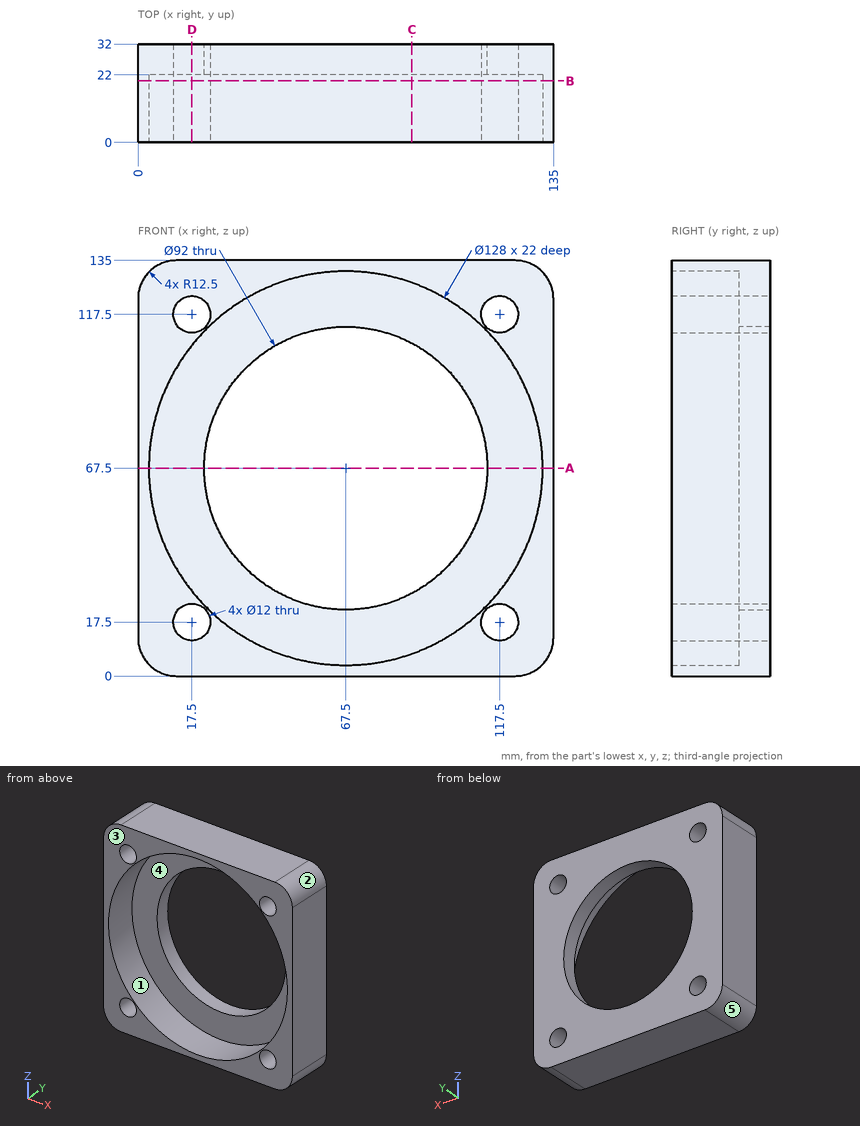
Check sheet for the drawn part. Datum: minimum x, y, z corner. Units: mm. A direction names the side the tool comes from. Give positions to 0.01 mm unless a question says otherwise; leave off trailing zeros. Order: outer loops, then holes, each group sorted by start corner. A loop starts at its lowest first (then second) coordinate and runs counter-clockwise, first axis right, second up. Notation, with made-up numbers: (32, -35.75) -> (85, -35.75) arc R32 ccw to (85, -7.75) -> close; hole circle Ø10 at (2.25, 72.25). An arc over 180 degrees is marked (long way). Use a Markdown table: item, result.
1) Mould release check, pull along X, two halves, no side actions. Record for the marked faces 3, 4 and 5: pulls with the +X half, pulls with the -X half, needs draft (parallel to the pull), parting line crosses it, or undercut.
Results:
| item | result |
|---|---|
| face 3 | needs draft |
| face 4 | undercut |
| face 5 | pulls with the -X half |
2) Section check B-B, the plane y = 20. Record the boundary of the cut face in (x, z).
Results:
| item | result |
|---|---|
| outline | (0, 12.5) arc R12.5 ccw to (12.5, 0) -> (122.5, 0) arc R12.5 ccw to (135, 12.5) -> (135, 122.5) arc R12.5 ccw to (122.5, 135) -> (12.5, 135) arc R12.5 ccw to (0, 122.5) -> close; hole circle Ø128 at (67.5, 67.5); hole circle Ø12 at (17.5, 17.5); hole circle Ø12 at (17.5, 117.5); hole circle Ø12 at (117.5, 17.5); hole circle Ø12 at (117.5, 117.5) |
3) Material ranges on probe 1 along X at (y, z) = (22.5, 117.5); probe 2 along Z at (x, y) = (116, 13); probe 3 along X at (y, z) = (15.5, 67.5), recorded low to high.
Results:
| item | result |
|---|---|
| probe 1 | 0 to 11.5, 23.5 to 111.5, 123.5 to 135 |
| probe 2 | 0 to 11.69, 23.31 to 25.74, 109.26 to 111.69, 123.31 to 135 |
| probe 3 | 0 to 3.5, 131.5 to 135 |
4) Section check A-A, the plane z = 67.5. Record the boundary of the cut face in (x, y).
Results:
| item | result |
|---|---|
| outline | (0, 0) -> (3.5, 0) -> (3.5, 22) -> (21.5, 22) -> (21.5, 32) -> (0, 32) -> close; (113.5, 22) -> (131.5, 22) -> (131.5, 0) -> (135, 0) -> (135, 32) -> (113.5, 32) -> close |
5) Section check C-C, the plane x = 89. Record the boundary of the cut face in (y, z), then the cut area to 3 significant figures.
Results:
| item | result |
|---|---|
| outline | (0, 0) -> (32, 0) -> (32, 26.83) -> (22, 26.83) -> (22, 7.22) -> (0, 7.22) -> close; (0, 127.78) -> (22, 127.78) -> (22, 108.17) -> (32, 108.17) -> (32, 135) -> (0, 135) -> close |
| area | 854 mm² |
6) Tool access check on the marked faces 1 and 2. Record the directions out of +Z, -Z, +X, -X, +Y, -Y that give a thin tool (end or side, any length) a straight path to the whole face; none if there is none.
Results:
| item | result |
|---|---|
| face 1 | -Y |
| face 2 | +Z, +X, +Y, -Y |
7) Depth check by flat-ended pin: pin 1 Ø9.5 at (x, z) = (17.5, 17.5) entering from +Y; pin 2 Ø12 at (x, z) = (97.5, 111) entering from -Y. Enter the tip coordinate at first touch or a pass-through.
Results:
| item | result |
|---|---|
| pin 1 | through |
| pin 2 | y = 22 |
8) Section check D-D, the plane x = 17.5. Record the boundary of the cut face in (y, z), then the cut area to 3 significant figures.
Results:
| item | result |
|---|---|
| outline | (0, 0) -> (32, 0) -> (32, 11.5) -> (0, 11.5) -> close; (0, 23.5) -> (32, 23.5) -> (32, 111.5) -> (0, 111.5) -> (0, 107.45) -> (22, 107.45) -> (22, 27.55) -> (0, 27.55) -> close; (0, 123.5) -> (32, 123.5) -> (32, 135) -> (0, 135) -> close |
| area | 1,790 mm² |
